The listing builds one solid part. Answer for the finished solid, in the listing's coordinates (mm). Coordinates: 2 decimals unless noted, no trailing zeros. Order: outer loops, then holes, each group sorted by start corner. A loop starts at its lowest first (then second) coordinate and runs counter-clockwise, first axis right, second up. Notation, with made-up numbers: (86.25, 10.25) - (95.25, 10.25) arc R5 ccw to (95.25, 14.25) - close; hole circle Ø2 at (-12, 23.25). An arc over 180 degrees is marked (long way). One line per item, written item: value. Start each with the question number.
```python
from build123d import *

# Parameters (mm, degrees)
SKETCH1_R          = 12.5
BASE_EXTRUDE_DEPTH = 15
SKETCH2_OUTSIDE_W  = 298.754
SKETCH2_OUTSIDE_H  = 304.43
SKETCH2_OUTSIDE_R  = 17.5
CUT_EXTRUDE1_DEPTH = 33.179208695
CUT_EXTRUDE1_DRAFT = -75
SKETCH3_OUTSIDE_W  = 298.754
SKETCH3_OUTSIDE_H  = 304.43
SKETCH3_OUTSIDE_R  = 17.5
CUT_EXTRUDE2_DEPTH = 33.179208695
CUT_EXTRUDE2_DRAFT = -75
CHAMFER1_SIZE      = 1.521428571


with BuildPart() as part:
    # Sketch1 → Base-Extrude (new body)
    with BuildSketch(Plane.XY):
        Polygon((0.084573131, 21.499833659), (-18.577115561, 10.823159309), (-18.661688692, -10.67667435), (-0.084573131, -21.499833659), (18.577115561, -10.823159309), (18.661688692, 10.67667435), align=None)
        Circle(SKETCH1_R, mode=Mode.SUBTRACT)
    extrude(amount=BASE_EXTRUDE_DEPTH)


with BuildPart() as cut_extrude1_tool:
    # Sketch2 outside → Cut-Extrude1 (with draft: the straight prism first)
    with BuildSketch(Plane(origin=(0, 0, 0), x_dir=(-1, 0, 0), z_dir=(0, 0, -1))):
        Rectangle(SKETCH2_OUTSIDE_W, SKETCH2_OUTSIDE_H)
        Circle(SKETCH2_OUTSIDE_R, mode=Mode.SUBTRACT)
    extrude(amount=-CUT_EXTRUDE1_DEPTH)
    # Cut-Extrude1: the draft: its side faces are tilted about the plane it starts from
    cut_extrude1_sides = [cut_extrude1_tool.faces().sort_by_distance(p)[0] for p in [
        (0, -152.215, 16.589604347),
        (-149.377, 0, 16.589604347),
        (0, 152.215, 16.589604347),
        (149.377, 0, 16.589604347),
        (17.5, 0, 16.589604347),
    ]]
    draft(cut_extrude1_sides, Plane(origin=(0, 0, 0), x_dir=(-1, 0, 0), z_dir=(0, 0, -1)), CUT_EXTRUDE1_DRAFT)


with BuildPart() as part_1:
    add(part.part)

    # Cut-Extrude1: cut by cut_extrude1_tool
    add(cut_extrude1_tool.part, mode=Mode.SUBTRACT)


with BuildPart() as cut_extrude2_tool:
    # Sketch3 outside → Cut-Extrude2 (with draft: the straight prism first)
    with BuildSketch(Plane.XY.offset(15)):
        Rectangle(SKETCH3_OUTSIDE_W, SKETCH3_OUTSIDE_H)
        Circle(SKETCH3_OUTSIDE_R, mode=Mode.SUBTRACT)
    extrude(amount=-CUT_EXTRUDE2_DEPTH)
    # Cut-Extrude2: the draft: its side faces are tilted about the plane it starts from
    cut_extrude2_sides = [cut_extrude2_tool.faces().sort_by_distance(p)[0] for p in [
        (0, -152.215, -1.589604347),
        (149.377, 0, -1.589604347),
        (0, 152.215, -1.589604347),
        (-149.377, 0, -1.589604347),
        (-17.5, 0, -1.589604347),
    ]]
    draft(cut_extrude2_sides, Plane.XY.offset(15), CUT_EXTRUDE2_DRAFT)


with BuildPart() as part_2:
    add(part_1.part)

    # Cut-Extrude2: cut by cut_extrude2_tool
    add(cut_extrude2_tool.part, mode=Mode.SUBTRACT)

    # Chamfer1
    chamfer1_edges = [part_2.edges().sort_by_distance(p)[0] for p in [
        (-12.5, 0, 0),
        (-12.5, 0, 15),
    ]]
    chamfer(chamfer1_edges, length=CHAMFER1_SIZE)


solid = part_2.part
```
(1) Consider probe 1 along X at (y, z) = (8, 13.75); probe 2 along Y at (x, z) = (5, 9.5); probe 3 along X at (y, z) = (-4, 14). Determine where each line is inside the solid, lowest interval first.
(2) The part is cut by section B-B on y = 0. Determine the outline of the cut face in (x, z), plus the area to 3 significant figures.
(3) Flat-ended cylindrical pins translate along their axes: pin 1 Ø1 at (y, z) = (-1, 10.5) entering from +X; pin 2 Ø1.5 at (x, z) = (-1, 11) entering from -Y; pin 3 Ø4 at (x, z) = (9, 12) entering from +Y; pin 4 Ø1 at (x, y) = (10, -6) entering from +Z. Find the tip coordinate at first contact, or state that the pin passes through.
(4) For a pull along X with two mould halves and no side action, classify faces 1 (the face through (-10, -7.7, 1.4)), 2 (the face through (9.116, -16.236, 7.399)), 3 (the face through (-8.16, -15.7, 0.05)) as pulls with the +X half, pulls with the -X half, needs draft (parallel to the pull), parting line crosses it, or undercut.
(5) The part is cut by section A-A on z = 12.75. Determine the outline of the cut face in (x, y).
Completed:
1. probe 1: x = -18.59 to -9.96, 9.96 to 18.65
1. probe 2: y = -18.59 to -11.46, 11.46 to 18.64
1. probe 3: x = -18.64 to -12.39, 12.39 to 18.6
2. outline: (-18.62, 0.3) - (-17.5, 0) - (-14.02, 0) - (-12.5, 1.52) - (-12.5, 13.48) - (-14.02, 15) - (-17.5, 15) - (-18.62, 14.7) - close; (12.5, 1.52) - (14.02, 0) - (17.5, 0) - (18.62, 0.3) - (18.62, 14.7) - (17.5, 15) - (14.02, 15) - (12.5, 13.48) - close
2. area: 178 mm2
3. pin 1: stops at x = 18.62
3. pin 2: stops at y = -21.4
3. pin 3: stops at y = 17.47
3. pin 4: passes through
4. face 1: undercut
4. face 2: pulls with the +X half
4. face 3: parting line crosses it
5. outline: (-18.66, -10.68) - (-0.08, -21.5) - (18.58, -10.82) - (18.66, 10.68) - (0.08, 21.5) - (-18.58, 10.82) - close; hole circle Ø25 at (0, 0)
